from build123d import *

# Parameters (mm, degrees)
BASE_BLOCK_50MM_DEPTH         = 50
STEP_BOSS_SKETCH_W            = 50
STEP_BOSS_SKETCH_H            = 55
STEP_BOSS_10MM_DEPTH          = 10
STEP_CUT_SKETCH_W             = 50
STEP_CUT_SKETCH_H             = 55
STEP_CUT_10MM_DEPTH           = 10
UPRIGHT_PAD_SKETCH_W          = 50
UPRIGHT_PAD_SKETCH_H          = 55
UPRIGHT_PAD_5MM_DEPTH         = 5
ARCH_BOSS_15MM_DEPTH          = 15
UPPER_BLOCK_SKETCH_W          = 50
UPPER_BLOCK_SKETCH_H          = 20
UPPER_BLOCK_10MM_DEPTH        = 10
BASE_SEMICIRCULAR_NOTCH_DEPTH = 15
ARCH_SEMICIRCULAR_CUT_DEPTH   = 25
SUPPORT_RIB_30MM_DEPTH        = 30
RIB_TRIM_CUT_20MM_DEPTH       = 20


with BuildPart() as part:
    # Base Profile Sketch → Base Block 50mm (new body)
    with BuildSketch(Plane.XY):
        Polygon((0, 0), (0, 55), (10, 55), (10, 35), (75, 35), (75, 10), (10, 10), (10, 0), align=None)
    extrude(amount=BASE_BLOCK_50MM_DEPTH)

    # Step Boss Sketch → Step Boss 10mm (add)
    with BuildSketch(Plane.ZY):
        with Locations((25, 27.5)):
            Rectangle(STEP_BOSS_SKETCH_W, STEP_BOSS_SKETCH_H)
    extrude(amount=STEP_BOSS_10MM_DEPTH)

    # Step Cut Sketch → Step Cut 10mm (cut)
    with BuildSketch(Plane.ZY.offset(10)):
        with Locations((25, 27.5)):
            Rectangle(STEP_CUT_SKETCH_W, STEP_CUT_SKETCH_H)
    extrude(amount=-STEP_CUT_10MM_DEPTH, mode=Mode.SUBTRACT)

    # Upright Pad Sketch → Upright Pad 5mm (add)
    with BuildSketch(Plane.ZY):
        with Locations((25, 27.5)):
            Rectangle(UPRIGHT_PAD_SKETCH_W, UPRIGHT_PAD_SKETCH_H)
    extrude(amount=UPRIGHT_PAD_5MM_DEPTH)

    # Arch Boss Sketch R25 → Arch Boss 15mm (add)
    with BuildSketch(Plane.ZY.offset(5)):
        with BuildLine():
            Line((0, 55), (50, 55))
            ThreePointArc((50, 55), (25, 80), (0, 55))
        make_face()
    extrude(amount=-ARCH_BOSS_15MM_DEPTH)

    # Upper Block Sketch → Upper Block 10mm (add)
    with BuildSketch(Plane(origin=(10, 0, 0), x_dir=(0, 0, -1), z_dir=(1, 0, 0))):
        with Locations((-25, 45)):
            Rectangle(UPPER_BLOCK_SKETCH_W, UPPER_BLOCK_SKETCH_H)
    extrude(amount=UPPER_BLOCK_10MM_DEPTH)

    # Base Notch Sketch Ø30 → Base Semicircular Notch (cut)
    with BuildSketch(Plane(origin=(10, 0, 0), x_dir=(0, 0, -1), z_dir=(1, 0, 0))):
        with BuildLine():
            Line((-40, 58), (-25, 58))
            Line((-25, 58), (-10, 58))
            ThreePointArc((-10, 58), (-25, 73), (-40, 58))
        make_face()
    extrude(amount=-BASE_SEMICIRCULAR_NOTCH_DEPTH, mode=Mode.SUBTRACT)

    # Arch Cut Sketch Ø30 → Arch Semicircular Cut (cut)
    with BuildSketch(Plane(origin=(0, 35, 0), x_dir=(1, 0, 0), z_dir=(0, 1, 0))):
        with BuildLine():
            Line((75, -10), (75, -40))
            ThreePointArc((75, -40), (60, -25), (75, -10))
        make_face()
    extrude(amount=-ARCH_SEMICIRCULAR_CUT_DEPTH, mode=Mode.SUBTRACT)

    # Rib Sketch → Support Rib 30mm (add)
    with BuildSketch(Plane.XY.offset(50)):
        Polygon((20, 55), (20, 35), (40, 35), align=None)
    extrude(amount=-SUPPORT_RIB_30MM_DEPTH)

    # Rib Trim Sketch → Rib Trim Cut 20mm (cut)
    with BuildSketch(Plane.XY.offset(50)):
        Polygon((20, 55), (20, 35), (40, 35), align=None)
    extrude(amount=-RIB_TRIM_CUT_20MM_DEPTH, mode=Mode.SUBTRACT)


solid = part.part
Check sheet for the modelled part. Datum: model origin and axes. Units: mm. A direction names the side the tool comes from. Give positions to 0.01 mm unless a question says otherwise; leave off trailing zeros. Loops run counter-clockwise (first coordinate to the right, second up) from the corner with the lowest first, then second, coordinate; pieces in that order, holes last. Notation, with made-up numbers: M 20,38 L 59,38 A16 cw 59,43 Z; hole C 18.5,17 d3. An arc over 180 degrees is marked long. Return JSON: item names as keys, results as strings. Group by question number.
1. Thickness scan on L1, parallel to Y at x = 11, z = 16; L2, parallel to X at y = 44, z = 3; L3, parallel to Z at x = 0.5, y = 68. Record the ranges inside material, lowest first.
2. Cross-section at D-D on x = 34.5. Record the boundary of the cut face in (y, z), plus the area to 4 significant figures.
3. Go/stop test with flat-tipped pins: pin 1 (4.5 mm diameter, centred on x = -1, z = 32, fed in from +Y); pin 2 (11 mm diameter, centred on y = 5.5, z = 29, fed in from +X); pin 3 (8 mm diameter, centred on y = 35.5, z = 21, fed in from +X); pin 4 (16 mm diameter, centred on y = 42.5, z = 43.5, fed in from +X). Record where each tip stops, or that it passes through.
4. Mould release check, pull along Z, two halves, no side actions. Record for faces 5 (the flat face through (30, 45, 25)), 6 (the cylindrical face through (3, 73, 25)), 7 (the flat face through (26, 27, 0)): released by +Z, released by -Z, zero draft, split by the parting line, or undercut.
5. Tool access check on faces 1 (the flat face through (20, 45, 40)), 2 (the flat face through (15, 55, 25)), 3 (the flat face through (10, 5, 25)), 4 (the flat face through (47, 35, 25)). Record the directions out of +Z, -Z, +X, -X, +Y, -Y that give a thin tool (end or side, any length) a straight path to the whole face; none if there is none.
6. Cross-section at C-C on y = 31.5. Record the boundary of the cut face in (x, z), plus the area to 3 significant figures.
7. Cross-section at A-A on z = 25. Record the boundary of the cut face in (x, y).
8. Cross-section at B-B on x = 63.5. Record the boundary of the cut face in (y, z).
Return value:
{
 "1": {"L1": "10 to 55", "L2": "-5 to 20", "L3": "3.65 to 13.82, 36.18 to 46.35"},
 "2": {"outline": "M 10,0 L 35,0 L 35,20 L 40.5,20 L 40.5,30 L 35,30 L 35,50 L 10,50 Z", "area": "1,305 mm^2"},
 "3": {"pin 1": "y = 79.54", "pin 2": "x = 61.82", "pin 3": "x = 62.29", "pin 4": "x = 75"},
 "4": {"face 5": "zero draft", "face 6": "undercut", "face 7": "released by -Z"},
 "5": {"face 1": "+Z, +X, +Y", "face 2": "+Z, -Z, +X, +Y", "face 3": "+Z, -Z, +X, -Y", "face 4": "+X, +Y"},
 "6": {"outline": "M -5,0 L 75,0 L 75,10 A15 cw 75,40 L 75,50 L -5,50 Z", "area": "3,650 mm^2"},
 "7": {"outline": "M -5,0 L 10,0 L 10,10 L 60,10 L 60,35 L 40,35 L 20,55 L 10,55 L 10,58 L -5,58 Z; M -5,73 L 10,73 L 10,80 L -5,80 Z"},
 "8": {"outline": "M 10,0 L 35,0 L 35,15.37 L 10,15.37 Z; M 10,34.63 L 35,34.63 L 35,50 L 10,50 Z"}
}
